Could you check a few things on this model? Use its own coordinates, in mm. A direction names the side the tool comes from. Coordinates: 2 decimals unless noted, no trailing zeros. Order: outer loops, then holes, each group sorted by start corner. A loop starts at its lowest first (then second) coordinate and runs counter-clockwise, first axis right, second up. Notation, with made-up numbers: (-38, 53.5) - (17, 53.5) arc R31 cw to (17, 83.5) - close; hole circle Ø9 at (3, -9). An arc over 180 degrees is marked (long way). Answer as CSV lines item,"result". Start each with the question number.
1. I want a section at D-D, the plane y = 2.75. List the corners of the cut face in (x, z) for me.
2. For pin 1 (11 mm diameter, centred on x = 51, y = -2, fed in from +Z); pin 2 (6 mm diameter, centred on y = -2, z = 19.5, fed in from -X); pin 3 (8 mm diameter, centred on x = 52, y = 0, fed in from +Z); pin 4 (1.5 mm diameter, centred on x = 30.5, y = -1.5, fed in from +Z), each with a flat end and sliding along its axis, tell me the tip position at first contact or that it passes through.
3. Thinking about a two-plate mould opening in Z: for faces 6 (the face through (46, 0, 19)), 7 (the face through (13, -5, 3)), 8 (the face through (8, 7, 6)), which applies, released by +Z, released by -Z, zero draft, split by the parting line, or undercut?
4. I want a section at B-B, the plane z = 21. List the corners of the cut face in (x, y) for me, and give its area (3 significant figures).
5. I need wall thicknesses on probe 1 along Y at (x, z) = (52, 1.95); probe 2 along Z at (x, y) = (60.5, 6.5); probe 3 along X at (y, z) = (-5.25, 16.25). Which ranges of each line are inside material? Lowest first, please.
6. For faces 1 (the face through (40, 0, 12)), 2 (the face through (63, 0, 3)), 3 (the face through (31, 11, 7)), 4 (the face through (-5, 0, 3)), 5 (the face through (33, 0, 19)), which set-ups out of +Z, -Z, +X, -X, +Y, -Y let a thin tool reach every point of the face, with its end or its side?
7. I want a section at A-A, the plane x = 43.5. List the corners of the cut face in (y, z) for me, and give its area (3 significant figures).
8. I want a section at C-C, the plane y = -7.75. List the corners of the cut face in (x, z) for me, and give its area (3 significant figures).
from build123d import *

# Parameters (mm, degrees)
BASE_BLOCK_22X22_DEPTH    = 6
SQUARE_CUTOUT_10X10_DEPTH = 6
LINK_BODY_DEPTH           = 22
LINK_START                = -22
LINK_SLOT_DEPTH           = 22
END_START                 = -6
END_TAB_DEPTH             = 6
CROSS_HOLE_SKETCH_R       = 5
CROSS_HOLE_10_DEPTH       = 25


with BuildPart() as part:
    # Base Block Sketch → Base Block 22x22 (new body)
    with BuildSketch(Plane.XY):
        with BuildLine():
            Line((0, 11), (52, 11))
            ThreePointArc((52, 11), (63, 0), (52, -11))
            Line((52, -11), (0, -11))
            ThreePointArc((0, -11), (-11, 0), (0, 11))
        make_face()
    extrude(amount=BASE_BLOCK_22X22_DEPTH)

    # Square Cutout Sketch → Square Cutout 10x10 (cut)
    with BuildSketch(Plane.XY.offset(6)):
        with BuildLine():
            Line((0, 5), (25, 5))
            ThreePointArc((25, 5), (30, 0), (25, -5))
            Line((25, -5), (0, -5))
            ThreePointArc((0, -5), (-5, 0), (0, 5))
        make_face()
    extrude(amount=-SQUARE_CUTOUT_10X10_DEPTH, mode=Mode.SUBTRACT)

    # Link Profile Sketch → Link Body (add)
    with BuildSketch(Plane.XZ.offset(11)):
        with BuildLine():
            Line((27, 6), (33, 6))
            Line((33, 6), (40, 6))
            Line((40, 6), (40, 19))
            Line((40, 19), (52, 19))
            Line((52, 19), (52, 25))
            Line((52, 25), (33, 25))
            Line((33, 25), (33, 19))
            Line((33, 19), (33, 12))
            ThreePointArc((33, 12), (31.242640687, 7.757359313), (27, 6))
        make_face()
    extrude(amount=-LINK_BODY_DEPTH)

    # Link Slot Sketch → Link Slot (cut)
    with BuildSketch(Plane(origin=(0, 0, 6), x_dir=(-1, 0, 0), z_dir=(0, 0, -1)).offset(LINK_START)):
        with BuildLine():
            Line((-27, 4.582575695), (-27, -4.582575695))
            ThreePointArc((-27, -4.582575695), (-30, 0), (-27, 4.582575695))
        make_face()
    extrude(amount=LINK_SLOT_DEPTH, mode=Mode.SUBTRACT)

    # End Tab Sketch → End Tab (add)
    with BuildSketch(Plane.XY.offset(25).offset(END_START)):
        with BuildLine():
            Line((52, 11), (52, -11))
            ThreePointArc((52, -11), (63, 0), (52, 11))
        make_face()
    extrude(amount=END_TAB_DEPTH)

    # Cross Hole Sketch → Cross Hole Ø10 (cut)
    with BuildSketch(Plane.XY.offset(25)):
        with Locations((52, 0)):
            Circle(CROSS_HOLE_SKETCH_R)
    extrude(amount=-CROSS_HOLE_10_DEPTH, mode=Mode.SUBTRACT)


solid = part.part
Solved:
1,outline,"(-10.65, 0) - (-4.18, 0) - (-4.18, 6) - (-10.65, 6) - close; (29.18, 0) - (47.82, 0) - (47.82, 6) - (40, 6) - (40, 19) - (47.82, 19) - (47.82, 25) - (33, 25) - (33, 12) arc R6 cw to (29.18, 6.41) - close; (56.18, 0) - (62.65, 0) - (62.65, 6) - (56.18, 6) - close; (56.18, 19) - (62.65, 19) - (62.65, 25) - (56.18, 25) - close"
2,pin 1,"stops at z = 25"
2,pin 2,"stops at x = 33"
2,pin 3,"passes through"
2,pin 4,"stops at z = 7.76"
3,face 6,"undercut"
3,face 7,"zero draft"
3,face 8,"released by +Z"
4,outline,"(33, -11) - (52, -11) arc R11 ccw to (52, 11) - (33, 11) - close; hole circle Ø10 at (52, 0)"
4,area,"530 mm2"
5,probe 1,"y = -11 to -5, 5 to 11"
5,probe 2,"z = 0 to 6, 19 to 25"
5,probe 3,"x = 33 to 40"
6,face 1,"+X, +Y, -Y"
6,face 2,"+Z, -Z, +X"
6,face 3,"+Z, -Z, +X, -X, +Y"
6,face 4,"+Z, -Z"
6,face 5,"+Z, -X, +Y, -Y"
7,outline,"(-11, 0) - (11, 0) - (11, 6) - (-11, 6) - close; (-11, 19) - (11, 19) - (11, 25) - (-11, 25) - close"
7,area,"264 mm2"
8,outline,"(-7.81, 0) - (59.81, 0) - (59.81, 6) - (40, 6) - (40, 19) - (59.81, 19) - (59.81, 25) - (33, 25) - (33, 12) arc R6 cw to (27, 6) - (-7.81, 6) - close"
8,area,"665 mm2"
